Input: part model. Units: mm. Frame: model coordinates. Face numbers are marked on the shaded views. Coordinates: 2 decimals unless noted, no trailing zeros. Write each loop counter-clockwise with the first axis right and the second up, starting at its lowest first coordinate (ties: lowest second). Pieces come first, ordered by that corner, then holes. Notation, with made-up numbers: M -5.75,61.25 L 40.25,61.25 A29 ccw 40.25,82.25 Z; hole C 47,14.5 d7. An arc over 180 degrees is marked long. Write each question's results on one line, items separated by ' | '. Start each with the question number.
1. Ray query, probe 1 along Y at (x, z) = (12.5, -2.25); probe 2 along X at (y, z) = (-23.5, 2); probe 3 along X at (y, z) = (-10.5, -2). Return the intervals inside material, ascending.
2. Pull-direction query (Z, two-part tool) for the marked faces 1, 2 and 3; classes: +Z half, -Z half, draft (parallel to the pull), parting line (faces both ways), or undercut.
3. Section query A-A, the plane z = 0. Output: boundary loops of the cut face in (x, y), and give its area (3 significant figures).
4. Section query B-B, the plane y = -4. Count the separate pieces of the cut face and the enclosed holes in it, and give its area (3 significant figures).
5. First-contact query: pin 1 (8.5 mm diameter, centred on x = 25, z = 0, fed in from -Y); pin 2 (3 mm diameter, centred on y = 26, z = 1, fed in from +X); pin 3 (9 mm diameter, centred on x = 25, z = 0, fed in from +Y). Flat tips, straight axial feed; report the tip coordinate or a pass-through.
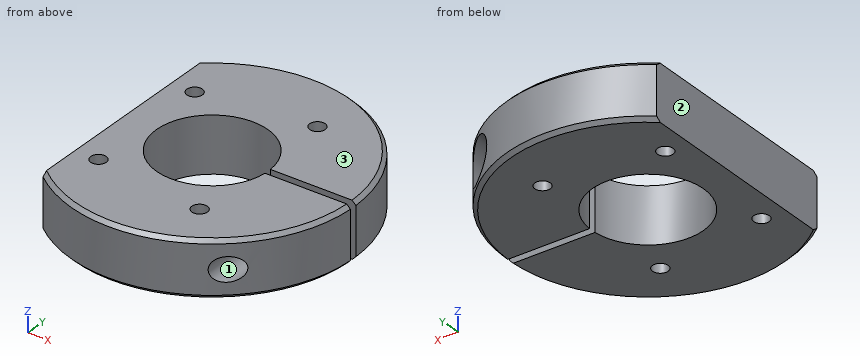
```python
from build123d import *

# Parameters (mm, degrees)
EXTRUDE_1_DEPTH              = 15
CUT_EXTRUDE_1_DEPTH          = 56.794264938
SKETCH_3_W                   = 15
SKETCH_3_H                   = 15
HOLE_WIZARD_4_2_4_2_1_D      = 4.2
SKETCH_6_W                   = 2.5
SKETCH_6_H                   = 37
HOLE_WIZARD_M6_1_D           = 6.5
HOLE_WIZARD_M6_1_DEPTH       = 70.615180295
HOLE_WIZARD_M6_1_CBORE_D     = 11
HOLE_WIZARD_M6_1_CBORE_DEPTH = 24.615180295
CHAMFER_1_SIZE               = 1


with BuildPart() as part:
    # 草图1 → 凸台-拉伸1 (new body)
    with BuildSketch(Plane(origin=(0, 0, -7.5), x_dir=(-1, 0, 0), z_dir=(0, 0, -1))):
        with BuildLine():
            Line((24, -29.461839725), (24, 29.461839725))
            ThreePointArc((24, 29.461839725), (-38, 0), (24, -29.461839725))
        make_face()
    extrude(amount=-EXTRUDE_1_DEPTH)

    # 草图2 → 切除-拉伸1 (cut, through all)
    with BuildSketch(Plane.XY.offset(7.5)):
        with BuildLine():
            Line((37.986839826, 1), (14.966629547, 1))
            ThreePointArc((14.966629547, 1), (15, 0), (14.966629547, -1))
            Line((14.966629547, -1), (37.986839826, -1))
            ThreePointArc((37.986839826, -1), (38, 0), (37.986839826, 1))
        make_face()
    extrude(amount=-CUT_EXTRUDE_1_DEPTH, mode=Mode.SUBTRACT)

    # 草图3 → 切除-旋转1 (revolve, cut)
    with BuildSketch(Plane.XZ):
        with Locations((7.5, 0)):
            Rectangle(SKETCH_3_W, SKETCH_3_H)
    revolve(axis=Axis((0, 0, 7.5), (0, 0, -1)), mode=Mode.SUBTRACT)

    # Ø4.2 (4.2) 直径孔1 (through all)
    with Locations(Plane.XY.offset(7.5)):
        with Locations((-17.67766953, -17.67766953), (-17.67766953, 17.67766953), (12.5, 21.650635095), (12.5, -21.650635095)):
            Hole(HOLE_WIZARD_4_2_4_2_1_D / 2)

    # 草图6 → Ø5.0 (5) 直径孔1 (revolve, cut)
    with BuildSketch(Plane(origin=(25, -1, 0), x_dir=(0, 0, 1), z_dir=(1, 0, 0))):
        with Locations((1.25, 18.5)):
            Rectangle(SKETCH_6_W, SKETCH_6_H)
    revolve(axis=Axis((25, 5.35, 0), (0, -1, 0)), mode=Mode.SUBTRACT)

    # M6 六角头螺栓的柱形沉头孔1
    with Locations(Plane(origin=(0, 32.615180295, 0), x_dir=(1, 0, 0), z_dir=(0, 1, 0))):
        with Locations((25, 0)):
            CounterBoreHole(HOLE_WIZARD_M6_1_D / 2, HOLE_WIZARD_M6_1_CBORE_D / 2, HOLE_WIZARD_M6_1_CBORE_DEPTH, depth=HOLE_WIZARD_M6_1_DEPTH)

    # 倒角1
    chamfer_1_edges = [part.edges().sort_by_distance(p)[0] for p in [
        (15.856449862, -34.533650224, 7.5),
        (15.856449862, 34.533650224, -7.5),
        (15.856449862, 34.533650224, 7.5),
        (15.856449862, -34.533650224, -7.5),
    ]]
    chamfer(chamfer_1_edges, length=CHAMFER_1_SIZE)


solid = part.part
```
Answer:
1) probe 1: -35.89 to -23.75, -19.55 to -8.29, 8.29 to 19.55, 23.75 to 35.89 | probe 2: -24 to 11.51, 13.49 to 22.44, 27.56 to 29.86 | probe 3: -24 to -10.71, 10.71 to 22.44, 27.56 to 36.52
2) face 1: undercut | face 2: draft | face 3: +Z half
3) outline: M -24,-29.46 A38 ccw 21.75,-31.16 L 21.75,-1 L 14.97,-1 A15 cw long 14.97,1 L 21.75,1 L 21.75,8 L 19.5,8 L 19.5,32.62 A38 ccw -24,29.46 Z; M 28.25,-25.42 A38 ccw 37.99,-1 L 28.25,-1 Z; M 28.25,1 L 37.99,1 A38 ccw 30.5,22.67 L 30.5,8 L 28.25,8 Z; hole C -17.68,-17.68 d4.2; hole C -17.68,17.68 d4.2; hole C 12.5,-21.65 d4.2; hole C 12.5,21.65 d4.2 | area: 2,710 mm^2
4) separate pieces: 2 | enclosed holes: 1 | area: 459 mm^2
5) pin 1: y = -31.83 | pin 2: x = 20.1 | pin 3: y = 8
